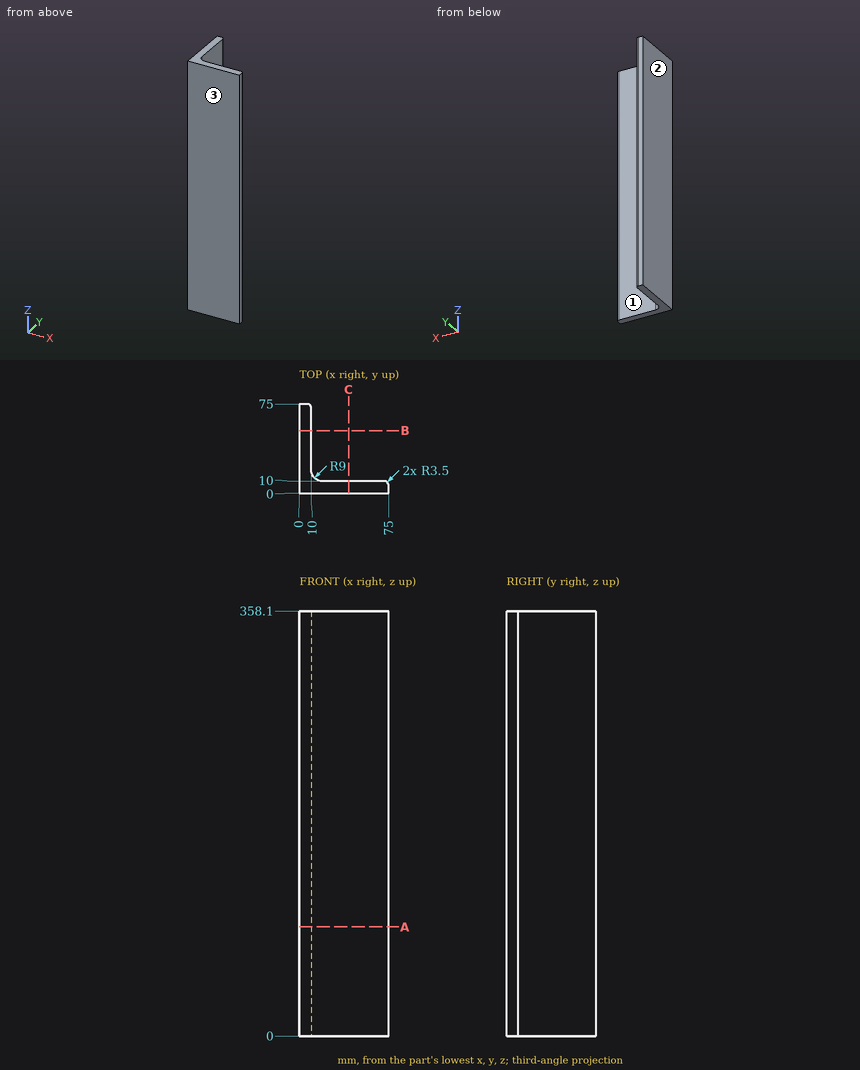
Design review of the part shown in the three views and the two pictorial views. Dimensions are in mm from the part's minimum x, y and z. Round coordinates to 2 decimals unless told otherwise and drop trailing zeros. Write each loop counter-clockwise with the first axis right and the second up, starting at its lowest first coordinate (ties: lowest second). Pieces come first, ordered by that corner, then holes. Notation, with made-up numbers: M 15,54.25 L 60,54.25 A36 cw 60,92.25 Z; hole C 17.25,-11 d4. An arc over 180 degrees is marked long. Use a Markdown table: item, result. Add a question column.
Q1. We need section B-B, the plane y = 52.5. State the section outline as (x, z) points.
Q2. The part is to be moulded in two halves that separate along Y. For the marked faces 1, 2 and 3, say which applies: pulls with the +Y half, pulls with the -Y half, needs draft (parallel to the pull), parting line crosses it, or undercut.
Q3. Insertion check: pin 1 (4 mm diameter, centred on y = 66.5, z = 46, fed in from +X); pin 2 (2 mm diameter, centred on x = 60, z = 121, fed in from +Y). Each pin has a flat end and moves straight along its axis. Give the tip position at first contact, or say it passes through.
Q4. To check wall thickness, follow line 1 (X direction, y = 49.5, z = 128); line 2 (Y direction, x = 7, z = 194). State the ranges of each line that lie inside material, in increasing order.
Q5. We need section A-A, the plane z = 92. State the section outline as (x, y) points.
Findings below:
| question | item | result |
|---|---|---|
| 1 | outline | M 0,0 L 10,0 L 10,358.1 L 0,358.1 Z |
| 2 | face 1 | pulls with the +Y half |
| 2 | face 2 | needs draft |
| 2 | face 3 | pulls with the -Y half |
| 3 | pin 1 | stops at x = 10 |
| 3 | pin 2 | stops at y = 10 |
| 4 | line 1 | x = 0 to 10 |
| 4 | line 2 | y = 0 to 74.96 |
| 5 | outline | M 0,0 L 75,0 L 75,6.5 A3.5 ccw 71.5,10 L 19,10 A9 cw 10,19 L 10,71.5 A3.5 ccw 6.5,75 L 0,75 Z |
